Input: part model. Units: mm. Frame: model coordinates. Coordinates: 2 decimals unless noted, no trailing zeros. Write each loop counter-clockwise with the first axis right and the second up, starting at its lowest first coordinate (ties: lowest second). Pieces come first, ordered by that corner, then holes. Notation, with made-up numbers: (-20.75, 9) - (24.25, 9) arc R26 cw to (24.25, 32) - close; hole circle Ø8 at (7.25, 8). An arc over 180 degrees is marked (long way). Put each result on its own line as item: value. Start each with the question number.
1. Cut plane B-B, the plane x = 0. Return loops of the section in (y, z).
2. Pin query (flat end, axial travel): pin 1 (8.5 mm diameter, centred on x = -127.28, z = -127.28, fed in from -Y); pin 2 (4 mm diameter, centred on x = -144.5, y = 4, fed in from +Z); pin 3 (5 mm diameter, centred on y = 3.5, z = -55, fed in from +X); pin 4 (5 mm diameter, centred on x = -53, y = 10.5, fed in from -Z). Return the tip coordinate at first contact, or that it passes through.
3. Cut plane A-A, the plane z = 0. Return loops of the section in (x, y).
4. Cut plane C-C, the plane y = 10. Count the separate pieces of the cut face and the enclosed holes in it, and give its area (3 significant figures).
5. Line query: line 1 (Z direction, x = 34, y = 11); line 2 (X direction, y = 4.25, z = 183); line 3 (Z direction, x = 12.5, y = 3.25). Output: solid intervals per line, ascending.
6. Cut plane D-D, the plane x = 127.5. Return loops of the section in (y, z), and give its area (3 significant figures).
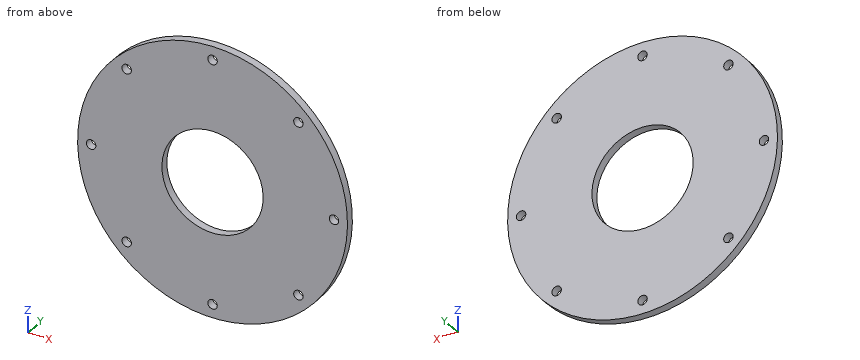
from build123d import *

# Parameters (mm, degrees)
SKETCH1_R                  = 200
SKETCH1_R_2                = 75
BOSS_EXTRUDE1_DEPTH        = 12
F_14_0_14_DIAMETER_HOLE1_D = 14


with BuildPart() as part:
    # Sketch1 → Boss-Extrude1 (new body)
    with BuildSketch(Plane(origin=(0, 0, 0), x_dir=(1, 0, 0), z_dir=(0, 1, 0))):
        with Locations(Location((0, 0, 0), (0, 0, 270))):
            Circle(SKETCH1_R)
        with Locations(Location((0, 0, 0), (0, 0, 270))):
            Circle(SKETCH1_R_2, mode=Mode.SUBTRACT)
    extrude(amount=BOSS_EXTRUDE1_DEPTH)

    # Ø14.0 (14) Diameter Hole1 (through all)
    with Locations(Plane(origin=(0, 12, 0), x_dir=(1, 0, 0), z_dir=(0, 1, 0))):
        with Locations((0, 180), (127.279220614, 127.279220614), (180, 0), (127.279220614, -127.279220614), (0, -180), (-127.279220614, -127.279220614), (-180, 0), (-127.279220614, 127.279220614)):
            Hole(F_14_0_14_DIAMETER_HOLE1_D / 2)


solid = part.part
Report:
1. outline: (0, -200) - (12, -200) - (12, -187) - (0, -187) - close; (0, -173) - (12, -173) - (12, -75) - (0, -75) - close; (0, 75) - (12, 75) - (12, 173) - (0, 173) - close; (0, 187) - (12, 187) - (12, 200) - (0, 200) - close
2. pin 1: passes through
2. pin 2: stops at z = 140.33
2. pin 3: stops at x = 192.99
2. pin 4: stops at z = -193.52
3. outline: (-200, 0) - (-187, 0) - (-187, 12) - (-200, 12) - close; (-173, 0) - (-75, 0) - (-75, 12) - (-173, 12) - close; (75, 0) - (173, 0) - (173, 12) - (75, 12) - close; (187, 0) - (200, 0) - (200, 12) - (187, 12) - close
4. separate pieces: 1
4. enclosed holes: 9
4. area: 107,000 mm^2
5. line 1: z = -197.09 to -66.85, 66.85 to 197.09
5. line 2: x = -80.69 to -6.32, 6.32 to 80.69
5. line 3: z = -199.61 to -73.95, 73.95 to 199.61
6. outline: (0, -154.09) - (12, -154.09) - (12, -134.28) - (0, -134.28) - close; (0, -120.28) - (12, -120.28) - (12, 120.28) - (0, 120.28) - close; (0, 134.28) - (12, 134.28) - (12, 154.09) - (0, 154.09) - close
6. area: 3,360 mm^2
